from build123d import *

# Parameters (mm, degrees)
SKETCH_1_R          = 1.5
EXTRUDE_1_DEPTH     = 10
SKETCH_2_R          = 3
M6X0_75P_DEPTH      = 14
SKETCH_3_R          = 1.1
EXTRUDE_3_DEPTH     = 20
CHAMFER_1_SIZE      = 0.5
SKETCH_4_W          = 2.061421144
SKETCH_4_H          = 7.488665512
CUT_EXTRUDE_1_DEPTH = 45.204072211


with BuildPart() as part:
    # 草图1 → 凸台-拉伸1 (new body)
    with BuildSketch(Plane(origin=(0, 0, 0), x_dir=(1, 0, 0), z_dir=(0, 1, 0))):
        with Locations(Location((0, 0, 0), (0, 0, 270))):
            Circle(SKETCH_1_R)
    extrude(amount=EXTRUDE_1_DEPTH)

    # 草图2 → M6X0.75P (add)
    with BuildSketch(Plane.XZ):
        with Locations(Location((0, 0, 0), (0, 0, 270))):
            Circle(SKETCH_2_R)
    extrude(amount=M6X0_75P_DEPTH)

    # 草图3 → 凸台-拉伸3 (add)
    with BuildSketch(Plane.XZ.offset(14)):
        with Locations(Location((0, 0, 0), (0, 0, 270))):
            Circle(SKETCH_3_R)
    extrude(amount=EXTRUDE_3_DEPTH)

    # 倒角1
    chamfer_1_edges = [part.edges().sort_by_distance(p)[0] for p in [
        (0, 0, 3),
        (0, -14, 3),
    ]]
    chamfer(chamfer_1_edges, length=CHAMFER_1_SIZE)

    # 草图4 → 切除-拉伸1 (cut, through all)
    with BuildSketch(Plane(origin=(0, 10, 0), x_dir=(1, 0, 0), z_dir=(0, 1, 0))):
        with Locations((3.430710572, 0.052409012)):
            Rectangle(SKETCH_4_W, SKETCH_4_H)
    cut_extrude_1 = extrude(amount=-CUT_EXTRUDE_1_DEPTH, mode=Mode.SUBTRACT)

    # 镜向1: 切除-拉伸1 across plane
    add(cut_extrude_1.mirror(Plane(origin=(0, 0, 0), x_dir=(0, 0, 1), z_dir=(1, 0, 0))), mode=Mode.SUBTRACT)


solid = part.part
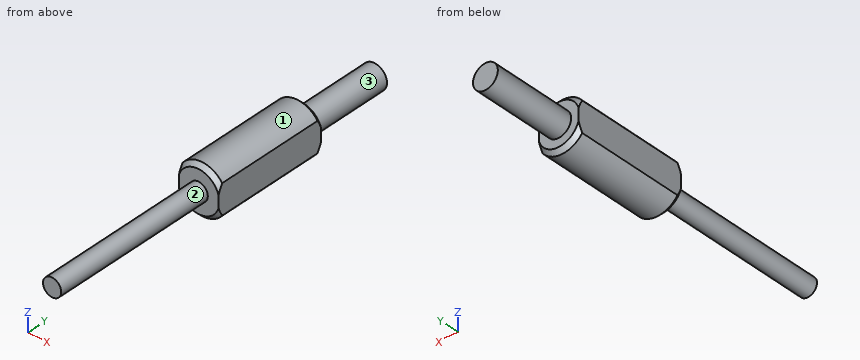
Model file for the job. Use its own axes, mm. Face numbers are marked on the shaded views. A direction names the side the tool comes from. Give positions to 0.01 mm unless a question says otherwise; leave off trailing zeros. Write each loop counter-clockwise with the first axis right and the second up, starting at its lowest first coordinate (ties: lowest second). Pieces come first, ordered by that corner, then holes. Notation, with made-up numbers: (31, 89.25) -> (77, 89.25) arc R17 cw to (77, 112.25) -> close; hole circle Ø5 at (-11, 9.5). An arc over 180 degrees is marked (long way). Write item = value, one per line.
(1) Flat gauge pins, fed straight in: P1, Ø1.5, axis at x = -2, y = -8.5, coming from the +Z side; P2, Ø2, axis at x = -1.5, y = -12, coming from the -Z side. Where does each tip first touch, or does it go through?
Determined:
P1 = 2.73
P2 = -2.96
(2) Tool access for the marked faces 1, 2 and 3: list every direction of +Z, -Z, +X, -X, +Y, -Y with a clear straight run to the whole face (end or side of a thin tool).
Determined:
face_1 = +Z, +Y, -Y
face_2 = -Y
face_3 = +Y
(3) Slice it at A-A, the plane x = 0. Give the cut face in (y, z).
Determined:
outline = (-34, -1.1) -> (-14, -1.1) -> (-14, -2.5) -> (-13.5, -3) -> (-0.5, -3) -> (0, -2.5) -> (0, -1.5) -> (10, -1.5) -> (10, 1.5) -> (0, 1.5) -> (0, 2.5) -> (-0.5, 3) -> (-13.5, 3) -> (-14, 2.5) -> (-14, 1.1) -> (-34, 1.1) -> close
(4) Probe line 1 along Y through (x, z) = (0.65, 1.25); line 2 along Y through (x, z) = (-1.05, -2); line 3 along Z through (x, y) = (1.5, -6.5). List the from-to ranges inside material, lowest first.
Determined:
line_1 = -14 to 10
line_2 = -14 to 0
line_3 = -2.6 to 2.6
(5) Slice it at B-B, the plane z = 0. Give the cut face in (x, y), then the cut area to 3 significant figures.
Determined:
outline = (-2.4, -14) -> (-1.1, -14) -> (-1.1, -34) -> (1.1, -34) -> (1.1, -14) -> (2.4, -14) -> (2.4, 0) -> (1.5, 0) -> (1.5, 10) -> (-1.5, 10) -> (-1.5, 0) -> (-2.4, 0) -> close
area = 141 mm2
(6) Slice it at D-D, the plane y = -11. Give the cut face in (x, z).
Determined:
outline = (-2.4, -1.8) arc R3 ccw to (2.4, -1.8) -> (2.4, 1.8) arc R3 ccw to (-2.4, 1.8) -> close
(7) Slice it at C-C, the plane y = -15.5. Give the cut face in (x, z), then the cut area to 3 significant figures.
Determined:
outline = circle Ø2.2 at (0, 0)
area = 3.80 mm2
